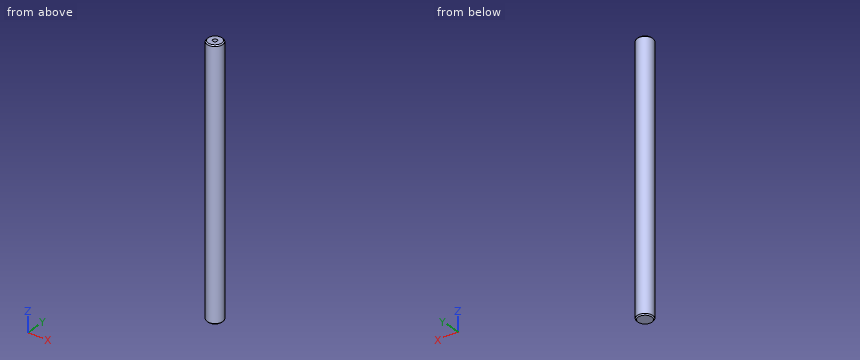
```python
from build123d import *

# Parameters (mm, degrees)
SKETCH1_R              = 15
BOSS_EXTRUDE1_DEPTH    = 500
CHAMFER1_SIZE          = 2
M10_TAPPED_HOLE1_D     = 8.5
M10_TAPPED_HOLE1_DEPTH = 24.5
M10_TAPPED_HOLE1_TIP   = 2.553657631


with BuildPart() as part:
    # Sketch1 → Boss-Extrude1 (new body)
    with BuildSketch(Plane.XY):
        Circle(SKETCH1_R)
    extrude(amount=BOSS_EXTRUDE1_DEPTH)

    # Chamfer1
    chamfer1_edges = [part.edges().sort_by_distance(p)[0] for p in [
        (-15, 0, 0),
        (-15, 0, 500),
    ]]
    chamfer(chamfer1_edges, length=CHAMFER1_SIZE)

    # M10 Tapped Hole1
    with Locations(Plane.XY.offset(500)):
        with Locations((0, 0)):
            Hole(M10_TAPPED_HOLE1_D / 2, depth=M10_TAPPED_HOLE1_DEPTH)
            with Locations((0, 0, -(M10_TAPPED_HOLE1_DEPTH + M10_TAPPED_HOLE1_TIP / 2))):  # 118° drill point
                Cone(0, M10_TAPPED_HOLE1_D / 2, M10_TAPPED_HOLE1_TIP, mode=Mode.SUBTRACT)


solid = part.part
```
The listing builds one solid part. Answer for the finished solid, in the listing's coordinates (mm). Give positions to 0.01 mm unless a question says otherwise; leave off trailing zeros. Order: outer loops, then holes, each group sorted by start corner. A loop starts at its lowest first (then second) coordinate and runs counter-clockwise, first axis right, second up.
Item 1: Find the intervals of material crossed by probe 1 along Y at (x, z) = (0, 480.75); probe 2 along Z at (x, y) = (-1, 4); probe 3 along Z at (x, y) = (1.75, -0.5), in increasing order.
From the geometry:
probe 1: y = -15 to -4.25, 4.25 to 15
probe 2: z = 0 to 475.42
probe 3: z = 0 to 474.04
Item 2: The part is cut by section A-A, the plane z = 392.5. Give the vertices of the cut face in (x, y).
From the geometry:
outline: circle Ø30 at (0, 0)
Item 3: Given pin 1 Ø1.5 at (x, z) = (1.5, 328.5) entering from +Y; pin 2 Ø1.5 at (y, z) = (7, 388.5) entering from +X; pin 3 Ø2 at (y, z) = (-10, 330) entering from -X, each flat-ended and moving along its own axis, determine where each tip first touches the part or whether it passes through.
From the geometry:
pin 1: stops at y = 14.98
pin 2: stops at x = 13.64
pin 3: stops at x = -12
